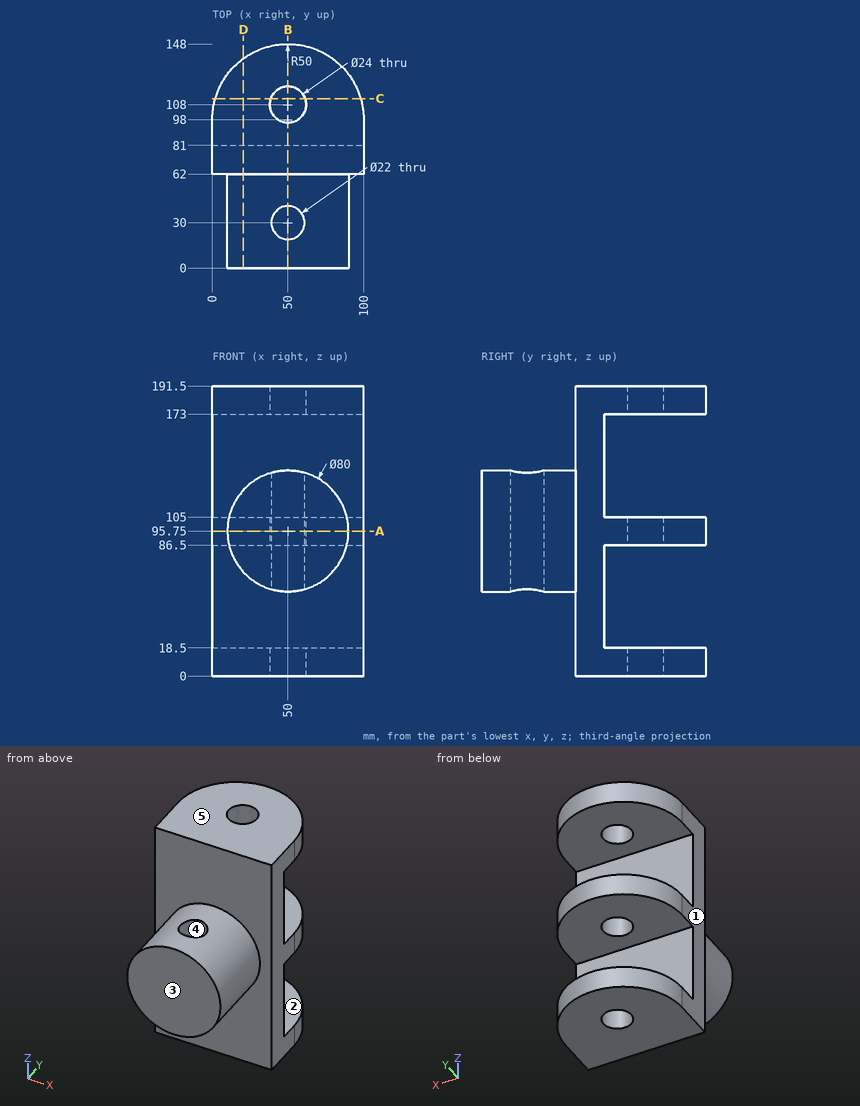
Answer from the drawing. Dimensions are ordinates in mm from the lowest x, y and z of the part. A direction names the side the tool comes from. Coordinates: 2 decimals unless noted, no trailing zeros. Loops run counter-clockwise (first coordinate to the right, second up) from the corner with the lowest first, then second, coordinate; pieces in that order, holes last. Notation, with made-up numbers: (-33, 31.25) -> (-9, 31.25) arc R33 cw to (-9, 63.25) -> close; hole circle Ø4 at (-9.75, -19.5). An arc over 180 degrees is marked (long way). Return JSON: item names as keys, results as strings.
Item 1: Flat-ended cylindrical pins translate along their axes: P1, Ø1, axis at x = 78, y = 43.5, coming from the +Z side; P2, Ø1, axis at x = 38.5, z = 51, coming from the +Y side; P3, Ø2, axis at x = 24.5, y = 21.5, coming from the -Z side. Find the tip coordinate at first contact, or state that the pin passes through.
Answers:
{"P1": "stops at z = 124.8", "P2": "stops at y = 81", "P3": "stops at z = 64.13"}
Item 2: Find the intervals of material crossed by probe 1 along Z at (x, y) = (43, 125); probe 2 along Y at (x, z) = (50, 85); probe 3 along Y at (x, z) = (55, 92), in increasing order.
Answers:
{"probe 1": "z = 0 to 18.5, 86.5 to 105, 173 to 191.5", "probe 2": "y = 0 to 19, 41 to 81", "probe 3": "y = 0 to 20.2, 39.8 to 97.09, 118.91 to 147.75"}
Item 3: Find section A-A (z = 95.75). Determine the outline of the cut face in (x, y).
Answers:
{"outline": "(0, 62) -> (10, 62) -> (10, 0) -> (90, 0) -> (90, 62) -> (100, 62) -> (100, 98) arc R50 ccw to (0, 98) -> close; hole circle Ø24 at (50, 108); hole circle Ø22 at (50, 30)"}
Item 4: Find section C-C (y = 112). Determine the outline of the cut face in (x, z).
Answers:
{"outline": "(2, 0) -> (38.69, 0) -> (38.69, 18.5) -> (2, 18.5) -> close; (2, 86.5) -> (38.69, 86.5) -> (38.69, 105) -> (2, 105) -> close; (2, 173) -> (38.69, 173) -> (38.69, 191.5) -> (2, 191.5) -> close; (61.31, 0) -> (98, 0) -> (98, 18.5) -> (61.31, 18.5) -> close; (61.31, 86.5) -> (98, 86.5) -> (98, 105) -> (61.31, 105) -> close; (61.31, 173) -> (98, 173) -> (98, 191.5) -> (61.31, 191.5) -> close"}
Item 5: Find section D-D (x = 20.5). Determine the outline of the cut face in (y, z), plus the area to 3 significant figures.
Answers:
{"outline": "(0, 68.74) -> (62, 68.74) -> (62, 0) -> (138.37, 0) -> (138.37, 18.5) -> (81, 18.5) -> (81, 86.5) -> (138.37, 86.5) -> (138.37, 105) -> (81, 105) -> (81, 173) -> (138.37, 173) -> (138.37, 191.5) -> (62, 191.5) -> (62, 122.76) -> (0, 122.76) -> close", "area": "10,200 mm2"}
Item 6: For the marked faces 1 and 2, determine the directions among +Z, -Z, +X, -X, +Y, -Y from which every point of the face is accessible in a straight line to the end or side of a thin tool.
Answers:
{"face 1": "+Z, -Z, -X, +Y, -Y", "face 2": "+X, -X, +Y"}
Item 7: For a pull along Y with two mould halves and no side action, classify the marked faces 3, 4 and 5 as +Y half, -Y half, draft (parallel to the pull), parting line (faces both ways), or undercut.
Answers:
{"face 3": "-Y half", "face 4": "undercut", "face 5": "draft"}
Item 8: Find section B-B (x = 50). Count the separate pieces of the cut face and the enclosed holes in it, plus the area to 4 significant figures.
Answers:
{"separate pieces": "5", "enclosed holes": "0", "area": "9,225 mm2"}
